Here's how the part is built. I have some questions about the finished solid (model axes, mm). A direction names the side the tool comes from. Round coordinates to 2 decimals unless told otherwise and drop trailing zeros. Order: outer loops, then holes, each group sorted by start corner. A loop starts at its lowest first (then second) coordinate and runs counter-clockwise, first axis right, second up. Notation, with made-up numbers: (7, 59) - (42, 59) arc R9 ccw to (42, 68) - close; hole circle Ø2 at (-32, 55). An arc over 180 degrees is marked (long way). Answer as a JSON object with one key per item and string values.
```python
from build123d import *

# Parameters (mm, degrees)
LOWER_BODY_BLOCK_DEPTH = 20
UPRIGHT_START          = -60
UPRIGHT_WEB_DEPTH      = 60
UPPER_START            = -60
UPPER_BODY_BLOCK_DEPTH = 20
LIFTING_EYE_SKETCH_R   = 17.5
LIFTING_EYE_LUG_DEPTH  = 20


with BuildPart() as part:
    # Body Block Profile Sketch → Lower Body Block (new body)
    with BuildSketch(Plane(origin=(0, 0, 0), x_dir=(1, 0, 0), z_dir=(0, 1, 0))):
        with BuildLine():
            Line((20, -35), (35, -35))
            Line((35, -35), (35, 35))
            Line((35, 35), (-35, 35))
            Line((-35, 35), (-35, -35))
            Line((-35, -35), (-20, -35))
            ThreePointArc((-20, -35), (0, -15), (20, -35))
        make_face()
    extrude(amount=LOWER_BODY_BLOCK_DEPTH)

    # Upright Web Sketch → Upright Web (add)
    with BuildSketch(Plane(origin=(0, 20, 0), x_dir=(1, 0, 0), z_dir=(0, 1, 0)).offset(UPRIGHT_START)):
        with BuildLine():
            Line((-35, -35), (-20, -35))
            ThreePointArc((-20, -35), (0, -15), (20, -35))
            Line((20, -35), (35, -35))
            Line((35, -35), (35, -10))
            Line((35, -10), (-35, -10))
            Line((-35, -10), (-35, -35))
        make_face()
    extrude(amount=UPRIGHT_WEB_DEPTH)

    # Sketch2_2 → Upper Body Block (add)
    with BuildSketch(Plane(origin=(0, 0, 0), x_dir=(1, 0, 0), z_dir=(0, 1, 0)).offset(UPPER_START)):
        with BuildLine():
            Line((20, -35), (35, -35))
            Line((35, -35), (35, 35))
            Line((35, 35), (-35, 35))
            Line((-35, 35), (-35, -35))
            Line((-35, -35), (-20, -35))
            ThreePointArc((-20, -35), (0, -15), (20, -35))
        make_face()
    extrude(amount=UPPER_BODY_BLOCK_DEPTH)

    # Lifting Eye Sketch → Lifting Eye Lug (add)
    with BuildSketch(Plane(origin=(0, 0, -35), x_dir=(-1, 0, 0), z_dir=(0, 0, -1))):
        with BuildLine():
            Line((-35, 60), (-35, 20))
            Line((-35, 20), (35, 20))
            Line((35, 20), (35, 60))
            ThreePointArc((35, 60), (0, 95), (-35, 60))
        make_face()
        with Locations((0, 60)):
            Circle(LIFTING_EYE_SKETCH_R, mode=Mode.SUBTRACT)
    extrude(amount=-LIFTING_EYE_LUG_DEPTH)


solid = part.part
```
1. For P1, Ø22.5, axis at x = 12, z = -22, coming from the +Y side; P2, Ø5, axis at x = 20.5, y = -38.5, coming from the -Z side; P3, Ø12, axis at x = 12, y = 39, coming from the +Z side; P4, Ø12, axis at x = -3, y = -20, coming from the -Z side, each with a flat end and sliding along its axis, tell me the tip position at first contact or that it passes through.
Responses:
{"P1": "y = 94.99", "P2": "z = -35", "P3": "z = -15", "P4": "z = 10"}
2. Imagine slicing it at A-A (z = -25.5). List the corners of the cut face in (x, y) for me, plus the area to 3 significant figures.
Responses:
{"outline": "(-35, -60) - (35, -60) - (35, -40) - (-35, -40) - close; (-35, 0) - (35, 0) - (35, 60) arc R35 ccw to (-35, 60) - close; hole circle Ø35 at (0, 60)", "area": "6,560 mm2"}
3. Imagine slicing it at D-D (y = 56.5). List the corners of the cut face in (x, z) for me, plus the area to 3 significant figures.
Responses:
{"outline": "(-35, -35) - (-17.15, -35) - (-17.15, -15) - (-35, -15) - close; (17.15, -35) - (35, -35) - (35, -15) - (17.15, -15) - close", "area": "714 mm2"}
4. Imagine slicing it at B-B (x = 0). List the corners of the cut face in (y, z) for me.
Responses:
{"outline": "(-60, -35) - (-40, -35) - (-40, 10) - (0, 10) - (0, -35) - (42.5, -35) - (42.5, -15) - (20, -15) - (20, 15) - (-60, 15) - close; (77.5, -35) - (95, -35) - (95, -15) - (77.5, -15) - close"}
5. Imagine slicing it at C-C (z = -4.5). List the corners of the cut face in (x, y) for me, plus the area to 3 significant figures.
Responses:
{"outline": "(-35, -60) - (35, -60) - (35, -40) - (-35, -40) - close; (-35, 0) - (35, 0) - (35, 20) - (-35, 20) - close", "area": "2,800 mm2"}
6. If I drill on L1, parallel to Y at x = 0, z = -20.75; L2, parallel to Y at x = -7.5, z = 3; L3, parallel to Y at x = 11, z = -17, over which ranges is the centre line in solid material (lowest first)? Write a range as [from, to].
Responses:
{"L1": "[-60, -40], [0, 42.5], [77.5, 95]", "L2": "[-60, -40], [0, 20]", "L3": "[-60, -40], [0, 46.39], [73.61, 93.23]"}
7. For faces 1 (the face through (0, -20, 10)), 2 (the face through (0, 41, -15)), 3 (the face through (-35, -14, 15)), which set-ups out of +Z, -Z, +X, -X, +Y, -Y let a thin tool reach every point of the face, with its end or its side?
Responses:
{"face 1": "-Z, +X, -X", "face 2": "+Z, +X, -X, +Y", "face 3": "+Z, -Z, -X, +Y, -Y"}
8. Thinking about a two-plate mould opening in Y: for faces 4 (the face through (0, -40, -13)), 5 (the face through (3.794, 42.916, -25.14)), 6 (the face through (35, 1, 0)), 7 (the face through (0, -60, 0)), which applies, pulls with the +Y half, pulls with the -Y half, needs draft (parallel to the pull), parting line crosses it, or undercut?
Responses:
{"face 4": "undercut", "face 5": "undercut", "face 6": "needs draft", "face 7": "pulls with the -Y half"}
